Here's how the part is built. I have some questions about the finished solid (model axes, mm). Face numbers are marked on the shaded views. A direction names the side the tool comes from. Coordinates: 2 decimals unless noted, no trailing zeros. Write each loop counter-clockwise with the first axis right and the second up, starting at its lowest first coordinate (ties: lowest second). Pieces come first, ordered by that corner, then holes. Notation, with made-up numbers: (-1.75, 79) -> (48.25, 79) arc R24 ccw to (48.25, 105) -> close; hole circle Ø7 at (-21, 80.5). An arc over 180 degrees is marked (long way). Put each result on its own line as item: value. Start each with the question number.
Item 1: I need wall thicknesses on line 1 (X direction, y = 15, z = 0); line 2 (Z direction, x = 5, y = -11); line 3 (Y direction, x = -33.5, z = 22). Which ranges of each line are inside material? Lowest first, please. Write a range as [from, to].
Item 2: I want a section at C-C, the plane y = -52. List the corners of the cut face in (x, z) for me.
Item 3: I want a section at D-D, the plane z = 25.5. List the corners of the cut face in (x, y) for me.
Item 4: I want a section at B-B, the plane z = -4.5. List the corners of the cut face in (x, y) for me.
Item 5: I want a section at A-A, the plane x = 0. List the corners of the cut face in (y, z) for me.
Item 6: On a 3-axis mill with a long thin cutter (end or side, diameter ignored), from which of +Z, -Z, +X, -X, +Y, -Y can I reach the whole of each face in a straight line? I mean the marked faces 5, 6, 7 and 8. Say none if no direction works.
Item 7: For pin 1 (1 mm diameter, centred on y = -23, z = -12.5, fed in from -X); pin 2 (1.5 mm diameter, centred on y = -22.5, z = -8, fed in from +X); pin 3 (10 mm diameter, centred on x = -15, z = 42.5, fed in from -Y), each with a flat end and sliding along its axis, tell me the tip position at first contact or that it passes through.
Item 8: If we mould it in two halves opening along Z, with no side actions, what happens to the marked faces 1, 2, 3 and 4? For each: released by +Z, released by -Z, zero draft, split by the parting line, or undercut.
from build123d import *

# Parameters (mm, degrees)
BASE_PLATE_SKETCH_R     = 10.5
BASE_PLATE_DEPTH        = 21
ANGLED_WEB_48DEG_DEPTH  = 21
UPRIGHT_BLOCK_DEPTH     = 78
CORNER_FILLETS_R18_R    = 18
HALF_ROUND_CUT_24_REACH = 140.171


with BuildPart() as part:
    # Base Plate Sketch → Base Plate (new body)
    with BuildSketch(Plane(origin=(0, 0, 0), x_dir=(1, 0, 0), z_dir=(0, 1, 0))):
        with BuildLine():
            Line((-21, 0), (-21, 35))
            Line((-21, 35), (21, 35))
            Line((21, 35), (21, 0))
            ThreePointArc((21, 0), (0, -21), (-21, 0))
        make_face()
        with Locations(Location((0, 0, 0), (0, 0, 90))):
            Circle(BASE_PLATE_SKETCH_R, mode=Mode.SUBTRACT)
    extrude(amount=BASE_PLATE_DEPTH)

    # Angled Web Sketch → Angled Web 48deg (add)
    with BuildSketch(Plane(origin=(0, 0, -35), x_dir=(-1, 0, 0), z_dir=(0, 0, -1))):
        Polygon((77.725454791, -42), (77.725454791, -57), (-77.725454791, -57), (-77.725454791, -42), (-21, 21), (21, 21), align=None)
    extrude(amount=-ANGLED_WEB_48DEG_DEPTH)

    # Upright Block Sketch → Upright Block (add)
    with BuildSketch(Plane.XY.offset(-14)):
        Polygon((-77.725454791, -42), (-28, -42), (-28, -21), (28, -21), (28, -42), (77.725454791, -42), (77.725454791, -57), (-77.725454791, -57), align=None)
    extrude(amount=UPRIGHT_BLOCK_DEPTH)

    # Corner Fillets R18
    corner_fillets_r18_edges = [part.edges().sort_by_distance(p)[0] for p in [
        (-77.725454791, -49.5, 64),
        (77.725454791, -49.5, 64),
    ]]
    fillet(corner_fillets_r18_edges, radius=CORNER_FILLETS_R18_R)

    # Half-Round Cut Sketch → Half-Round Cut Ø24 (cut, up to next)
    with BuildSketch(Plane.XY.offset(64), mode=Mode.PRIVATE) as half_round_cut_24_sk1:
        with BuildLine():
            Line((-24, -57), (24, -57))
            ThreePointArc((24, -57), (0, -33), (-24, -57))
        make_face()
    half_round_cut_24_tool1 = extrude(half_round_cut_24_sk1.sketch, amount=-HALF_ROUND_CUT_24_REACH, mode=Mode.PRIVATE) & part.part
    add(half_round_cut_24_tool1.solids().sort_by_distance((0, -46.814084, 64))[0], mode=Mode.SUBTRACT)


solid = part.part
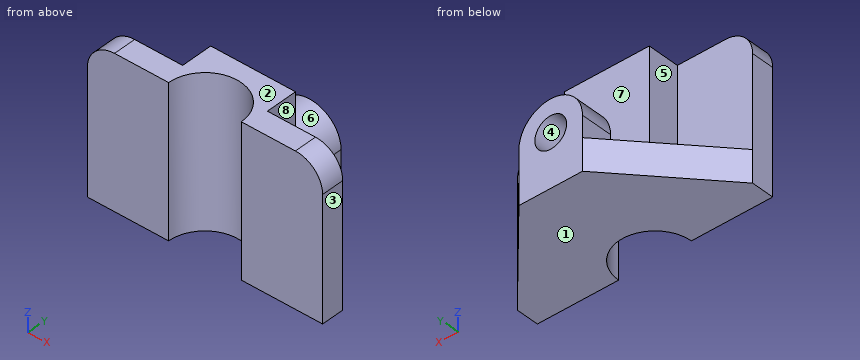
Calculated:
1. line 1: x = [-21, -10.5], [10.5, 21]
1. line 2: z = [-35, -14]
1. line 3: y = [-57, -42]
2. outline: (-77.73, -35) -> (-23.47, -35) -> (-23.47, 64) -> (-59.73, 64) arc R18 ccw to (-77.73, 46) -> close; (23.47, -35) -> (77.73, -35) -> (77.73, 46) arc R18 ccw to (59.73, 64) -> (23.47, 64) -> close
3. outline: (-77.73, -57) -> (-24, -57) arc R24 cw to (24, -57) -> (77.73, -57) -> (77.73, -42) -> (28, -42) -> (28, -21) -> (-28, -21) -> (-28, -42) -> (-77.73, -42) -> close
4. outline: (-77.73, -57) -> (-24, -57) arc R24 cw to (24, -57) -> (77.73, -57) -> (77.73, -42) -> (28, -42) -> (28, -21) -> (-28, -21) -> (-28, -42) -> (-77.73, -42) -> close; (-21, 0) -> (-9.49, 0) -> (-9.49, 21) -> (-21, 21) -> close; (9.49, 0) -> (21, 0) -> (21, 21) -> (9.49, 21) -> close
5. outline: (-33, -35) -> (21, -35) -> (21, -10.5) -> (0, -10.5) -> (0, -14) -> (-21, -14) -> (-21, 64) -> (-33, 64) -> close; (0, 10.5) -> (21, 10.5) -> (21, 21) -> (0, 21) -> close
6. face 5: +Z, -X, +Y
6. face 6: +Z, +Y
6. face 7: +Z, +X, -X
6. face 8: +Z, +X, +Y
7. pin 1: stops at x = -28
7. pin 2: stops at x = 28
7. pin 3: stops at y = -43.73
8. face 1: released by -Z
8. face 2: released by +Z
8. face 3: zero draft
8. face 4: undercut
